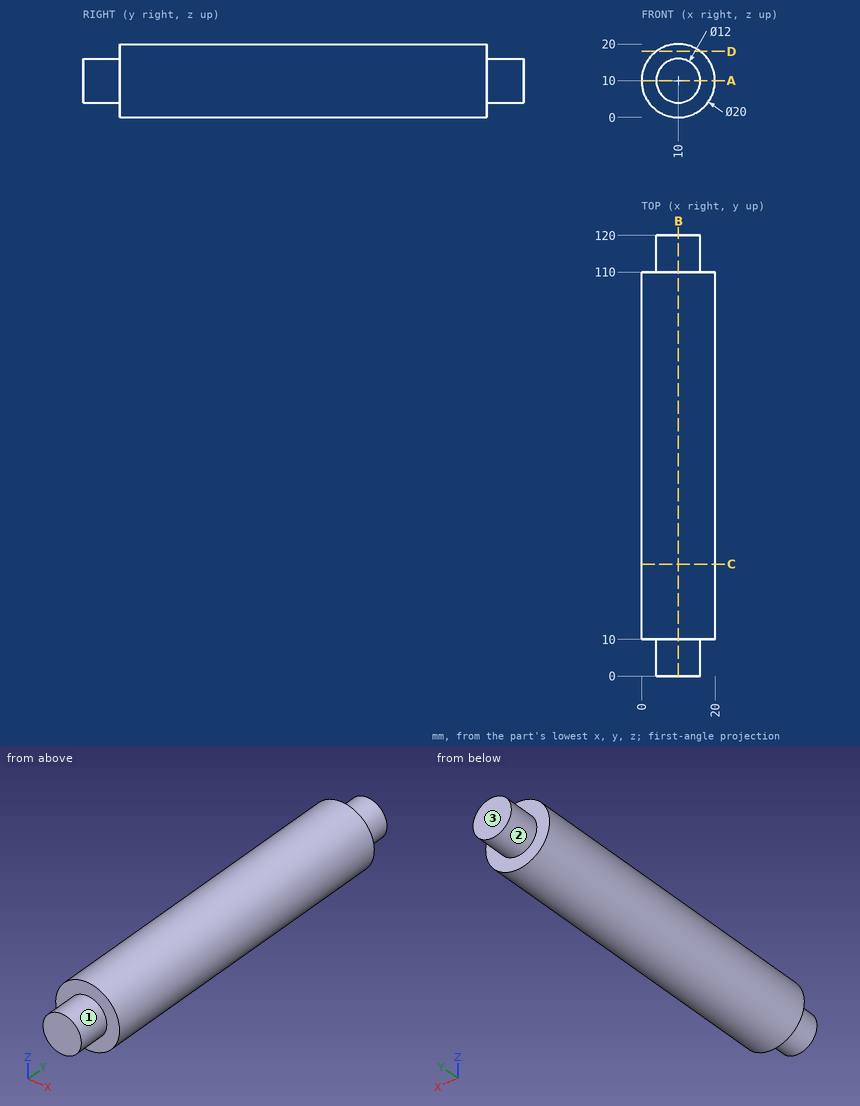
Here's the drawing with two shaded views (mm, measured from the low corner). I have some questions. A direction names the side the tool comes from. Coordinates: 2 decimals unless noted, no trailing zeros. Order: outer loops, then holes, each group sorted by start corner. A loop starts at its lowest first (then second) coordinate and runs counter-clockwise, first axis right, second up.
Q1. Will these pins go through, and if not, where does the flat tip stop? pin 1 (1.5 mm diameter, centred on y = 59, z = 17.5, fed in from +X); pin 2 (12 mm diameter, centred on x = 2.5, y = 51, fed in from -Z); pin 3 (2 mm diameter, centred on x = 17.5, y = 28.5, fed in from +Z).
Q2. Please list where these lines run through material, in increasing order: L1, parallel to Y at x = 14, z = 15.25; L2, parallel to Z at x = 9.5, y = 67; L3, parallel to X at y = 93.5, z = 10.25.
Q3. Suppose I cut it at C-C on y = 30.5. Please give me the cut outline in (x, z), and give its area (3 significant figures).
Q4. Suppose I cut it at B-B on x = 10. Please give me the cut outline in (y, z), and give its area (3 significant figures).
Q5. Suppose I cut it at A-A on z = 10. Please give me the cut outline in (x, y), and give its area (3 significant figures).
Q6. Which directions (+Z, -Z, +X, -X, +Y, -Y) give clear straight access to the entire face, cutting with the end or side of a thin tool? Please do the marked faces 1, 2 and 3.
Q7. Suppose I cut it at D-D on z = 18. Please give me the cut outline in (x, y).
Answer:
1. pin 1: stops at x = 17.38
1. pin 2: stops at z = 0.11
1. pin 3: stops at z = 17.6
2. L1: y = 10 to 110
2. L2: z = 0.01 to 19.99
2. L3: x = 0 to 20
3. outline: circle Ø20 at (10, 10)
3. area: 314 mm2
4. outline: (0, 4) - (10, 4) - (10, 0) - (110, 0) - (110, 4) - (120, 4) - (120, 16) - (110, 16) - (110, 20) - (10, 20) - (10, 16) - (0, 16) - close
4. area: 2,240 mm2
5. outline: (0, 10) - (4, 10) - (4, 0) - (16, 0) - (16, 10) - (20, 10) - (20, 110) - (16, 110) - (16, 120) - (4, 120) - (4, 110) - (0, 110) - close
5. area: 2,240 mm2
6. face 1: -Y
6. face 2: +Y
6. face 3: +Z, -Z, +X, -X, +Y
7. outline: (4, 10) - (16, 10) - (16, 110) - (4, 110) - close
